Drawing for the job (mm, zero at the part's lowest x, y, z). Give positions to 0.01 mm unless a question says otherwise; leave off trailing zeros. Order: outer loops, then holes, each group sorted by start corner. A loop starts at its lowest first (then second) coordinate and runs counter-clockwise, first axis right, second up. Notation, with made-up numbers: (13.5, 45) - (20.5, 45) arc R12 cw to (20.5, 63) - close; hole circle Ø10 at (48.5, 50.25). An arc over 180 degrees is marked (long way). One line per item, written item: value.
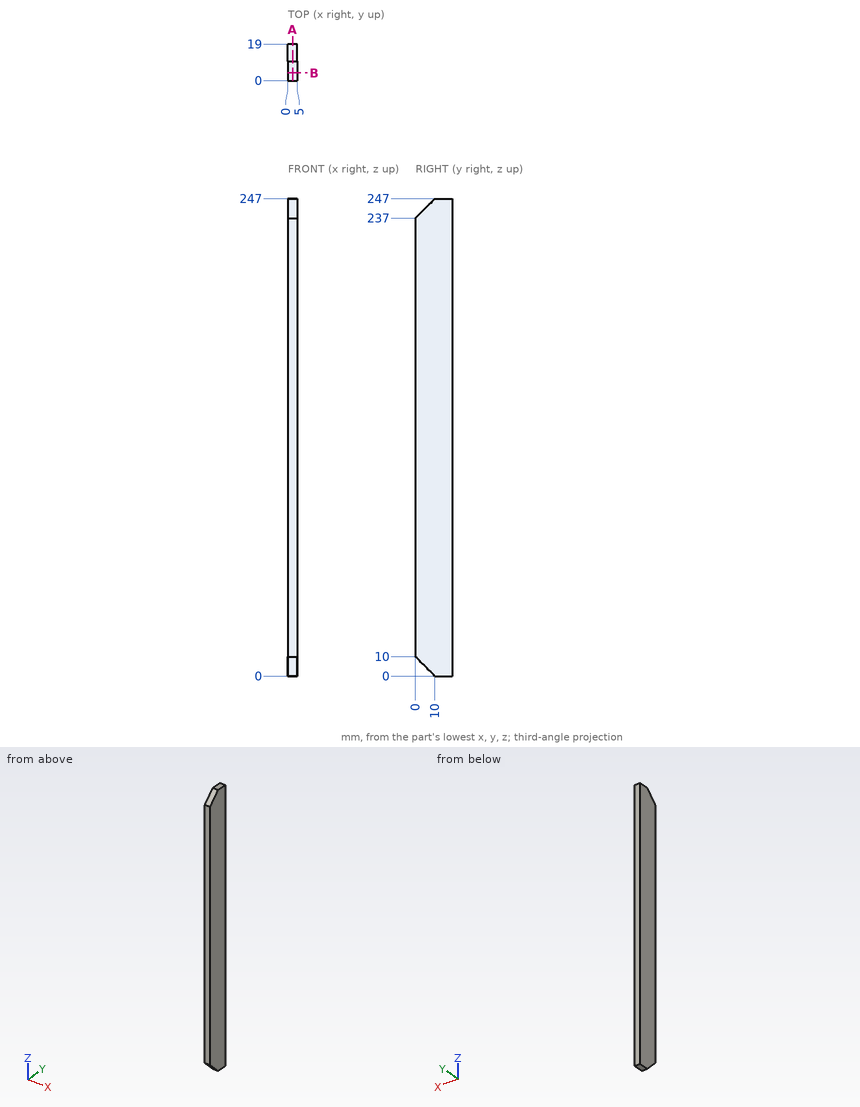
1) Cut at A-A, the plane x = 2.55. Give the cut face in (y, z).
Outcome:
outline: (0, 10) - (10, 0) - (19, 0) - (19, 247) - (10, 247) - (0, 237) - close
2) Cut at B-B, the plane y = 4. Give the cut face in (x, z), then the cut area to 4 significant figures.
Outcome:
outline: (0, 6) - (5, 6) - (5, 241) - (0, 241) - close
area: 1,175 mm^2
3) Drill centre lines: line 1 along Z through (x, y) = (0.6, 8); line 2 along Z through (x, y) = (0.35, 1). Where is each one in solid material? Low to high. Write a range as from..to.
Outcome:
line 1: z = 2..245
line 2: z = 9..238
4) Pin check, flat tip, straight feed: pin 1 (4 mm diameter, centred on y = 4, z = 66, fed in from -X). Stop position of the tip, or through.
Outcome:
pin 1: stops at x = 0
